```python
from build123d import *

# Parameters (mm, degrees)
BOSS_EXTRUDE1_DEPTH = 625


with BuildPart() as part:
    # Sketch1 → Boss-Extrude1 (new, symmetric)
    with BuildSketch(Plane.XY):
        with BuildLine():
            Line((-17, -25), (17, -25))
            ThreePointArc((17, -25), (22.656854249, -22.656854249), (25, -17))
            Line((25, -17), (25, 17))
            ThreePointArc((25, 17), (22.656854249, 22.656854249), (17, 25))
            Line((17, 25), (-17, 25))
            ThreePointArc((-17, 25), (-22.656854249, 22.656854249), (-25, 17))
            Line((-25, 17), (-25, -17))
            ThreePointArc((-25, -17), (-22.656854249, -22.656854249), (-17, -25))
        make_face()
        with BuildLine():
            Line((-17, 21), (17, 21))
            ThreePointArc((17, 21), (19.828427125, 19.828427125), (21, 17))
            Line((21, 17), (21, -17))
            ThreePointArc((21, -17), (19.828427125, -19.828427125), (17, -21))
            Line((17, -21), (-17, -21))
            ThreePointArc((-17, -21), (-19.828427125, -19.828427125), (-21, -17))
            Line((-21, -17), (-21, 17))
            ThreePointArc((-21, 17), (-19.828427125, 19.828427125), (-17, 21))
        make_face(mode=Mode.SUBTRACT)
    extrude(amount=BOSS_EXTRUDE1_DEPTH, both=True)


solid = part.part
```
The listing builds one solid part. Answer for the finished solid, in the listing's coordinates (mm). A direction names the side the tool comes from. Give positions to 0.01 mm unless a question says otherwise; leave off trailing zeros. Order: outer loops, then holes, each group sorted by start corner. A loop starts at its lowest first (then second) coordinate and runs counter-clockwise, first axis right, second up. Notation, with made-up numbers: (-1.75, 39.5) - (33.25, 39.5) arc R25 cw to (33.25, 55.5) - close; hole circle Ø3 at (13.5, 9). An arc over 180 degrees is marked (long way). Answer in a Markdown table with one row per item. Add a question column.
Q1. Which of the six approach directions +Z, -Z, +X, -X, +Y, -Y give full straight-line access (tool end or side, diameter ignored) to faces 5 (the flat face through (0, -25, 9)), 6 (the flat face through (21, 0, 9))?
Q2. The part is cut by section A-A (y = -7). Determine the outline of the cut face in (x, z).
Q3. For a pull along Y with two mould halves and no side action, classify faces 1 (the flat face through (0, -21, 9)), 2 (the flat face through (0, 25, 9)), 3 (the flat face through (-25, 0, 9)), 4 (the flat face through (0, 21, 9)) as released by +Y, released by -Y, zero draft, split by the parting line, or undercut.
Q4. Find the intervals of material crossed by line 1 along Y through (x, z) = (11, -216.5); line 2 along X through (y, z) = (18, -547), in increasing order. Write a range as [from, to].
Q5. Given P1, Ø2, axis at x = -17.5, z = -423, coming from the -Y side; P2, Ø1.5, axis at x = -18.5, z = -66, coming from the +Y side, each flat-ended and moving along its own axis, determine where each tip first touches the part or whether it passes through.
Q6. The part is cut by section C-C (z = 141). Determine the outline of the cut face in (x, y).
Determined:
| question | item | result |
|---|---|---|
| 1 | face 5 | +Z, -Z, +X, -X, -Y |
| 1 | face 6 | +Z, -Z |
| 2 | outline | (-25, -625) - (-21, -625) - (-21, 625) - (-25, 625) - close; (21, -625) - (25, -625) - (25, 625) - (21, 625) - close |
| 3 | face 1 | undercut |
| 3 | face 2 | released by +Y |
| 3 | face 3 | zero draft |
| 3 | face 4 | undercut |
| 4 | line 1 | y = [-25, -21], [21, 25] |
| 4 | line 2 | x = [-24.94, -20.87], [20.87, 24.94] |
| 5 | P1 | stops at y = -25 |
| 5 | P2 | stops at y = 24.96 |
| 6 | outline | (-25, -17) arc R8 ccw to (-17, -25) - (17, -25) arc R8 ccw to (25, -17) - (25, 17) arc R8 ccw to (17, 25) - (-17, 25) arc R8 ccw to (-25, 17) - close; hole (-21, -17) arc R4 ccw to (-17, -21) - (17, -21) arc R4 ccw to (21, -17) - (21, 17) arc R4 ccw to (17, 21) - (-17, 21) arc R4 ccw to (-21, 17) - close |
